```python
from build123d import *

# Parameters (mm, degrees)
SKETCH1_R           = 40
BOSS_EXTRUDE1_DEPTH = 40
M16_TAPPED_HOLE1_D  = 14


with BuildPart() as part:
    # Sketch1 → Boss-Extrude1 (new body)
    with BuildSketch(Plane.XY):
        with BuildLine():
            Line((-215.1, -380), (-173.1, -380))
            ThreePointArc((-173.1, -380), (-167.443145751, -377.656854249), (-165.1, -372))
            Line((-165.1, -372), (-165.1, -342))
            ThreePointArc((-165.1, -342), (-162.171067812, -334.928932188), (-155.1, -332))
            Line((-155.1, -332), (155.1, -332))
            ThreePointArc((155.1, -332), (162.171067812, -334.928932188), (165.1, -342))
            Line((165.1, -342), (165.1, -372))
            ThreePointArc((165.1, -372), (167.443145751, -377.656854249), (173.1, -380))
            Line((173.1, -380), (215.1, -380))
            Line((215.1, -380), (215.1, -74))
            Line((215.1, -74), (70.789255941, 70.632012878))
            ThreePointArc((70.789255941, 70.632012878), (0, 100), (-70.789255941, 70.632012878))
            Line((-70.789255941, 70.632012878), (-215.1, -74))
            Line((-215.1, -74), (-215.1, -380))
        make_face()
        Circle(SKETCH1_R, mode=Mode.SUBTRACT)
    extrude(amount=BOSS_EXTRUDE1_DEPTH)

    # M16 Tapped Hole1 (through all)
    with Locations(Plane.XY.offset(40)):
        with Locations((0, 70), (70, 0), (0, -70), (-70, 0)):
            Hole(M16_TAPPED_HOLE1_D / 2)


solid = part.part
```
Work out the finished part from the listing and answer in its coordinate system (mm). A direction names the side the tool comes from. Round coordinates to 2 decimals unless told otherwise and drop trailing zeros. Write each loop counter-clockwise with the first axis right and the second up, starting at its lowest first coordinate (ties: lowest second). Pieces come first, ordered by that corner, then holes. Notation, with made-up numbers: (-27.75, 26) - (2.25, 26) arc R20 cw to (2.25, 35) - close; hole circle Ø5 at (14, 55). An arc over 180 degrees is marked (long way). Return JSON: item names as keys, results as strings. Group by question number.
Q1. The part is cut by section B-B on y = -31.5. Write down the section's boundary in (x, z).
Q2. The part is cut by section D-D on x = 113. Write down the section's boundary in (y, z).
Q3. Each of these flat-tipped pins is pushed along its axis until it touches: pin 1 Ø6 at (x, z) = (63, 10) entering from +Y; pin 2 Ø1 at (y, z) = (51.5, 8.5) entering from +X; pin 3 Ø1.5 at (x, z) = (36, 30) entering from +Y; pin 4 Ø8.5 at (x, y) = (70, 0) entering from +Z. Where does it stop, or does it pass through?
Q4. The mould has two halves that part along X. Classify faces 1 (the cylindrical face through (162.09, -334.85, 19.72)), 2 (the flat face through (-3, -137, 0)), 3 (the flat face through (143.955, -2.696, 19.72)): released by +X, released by -X, zero draft, split by the parting line, or undercut.
Q5. The part is cut by section C-C on z = 25. Write down the section's boundary in (x, y).
Q6. The part is cut by section A-A on x = 0. Write down the section's boundary in (y, z).
Q7. Find the intervals of material crossed by L1, parallel to Y at x = 0, z = 17; L2, parallel to X at y = -353.5, z = 11; L3, parallel to Y at x = -9.5, z = 7, in increasing order.
Q8. For faces 4 (the cylindrical face through (0.91, -63.06, 19.72)), 5 (the flat face through (165.1, -357, 20)), determine the directions among +Z, -Z, +X, -X, +Y, -Y from which every point of the face is accessible in a straight line to the end or side of a thin tool.
Solved:
{
 "1": {"outline": "(-172.69, 0) - (-24.65, 0) - (-24.65, 40) - (-172.69, 40) - close; (24.65, 0) - (172.69, 0) - (172.69, 40) - (24.65, 40) - close"},
 "2": {"outline": "(-332, 0) - (28.33, 0) - (28.33, 40) - (-332, 40) - close"},
 "3": {"pin 1": "y = 80", "pin 2": "x = 90.38", "pin 3": "y = 93.58", "pin 4": "through"},
 "4": {"face 1": "undercut", "face 2": "zero draft", "face 3": "released by +X"},
 "5": {"outline": "(-215.1, -380) - (-173.1, -380) arc R8 ccw to (-165.1, -372) - (-165.1, -342) arc R10 cw to (-155.1, -332) - (155.1, -332) arc R10 cw to (165.1, -342) - (165.1, -372) arc R8 ccw to (173.1, -380) - (215.1, -380) - (215.1, -74) - (70.79, 70.63) arc R100 ccw to (-70.79, 70.63) - (-215.1, -74) - close; hole circle Ø14 at (-70, 0); hole circle Ø80 at (0, 0); hole circle Ø14 at (0, -70); hole circle Ø14 at (0, 70); hole circle Ø14 at (70, 0)"},
 "6": {"outline": "(-332, 0) - (-77, 0) - (-77, 40) - (-332, 40) - close; (-63, 0) - (-40, 0) - (-40, 40) - (-63, 40) - close; (40, 0) - (63, 0) - (63, 40) - (40, 40) - close; (77, 0) - (100, 0) - (100, 40) - (77, 40) - close"},
 "7": {"L1": "-332 to -77, -63 to -40, 40 to 63, 77 to 100", "L2": "-215.1 to -165.1, 165.1 to 215.1", "L3": "-332 to -38.86, 38.86 to 99.55"},
 "8": {"face 4": "+Z, -Z", "face 5": "+Z, -Z, -Y"}
}
